from build123d import *

# Parameters (mm, degrees)
SKETCH1_R           = 125
SKETCH1_R_2         = 110
BOSS_EXTRUDE1_DEPTH = 18
SKETCH2_R           = 175
SKETCH2_R_2         = 9
BOSS_EXTRUDE2_DEPTH = 15
CHAMFER1_SIZE       = 2
SKETCH3_R           = 67.5
CUT_EXTRUDE1_DEPTH  = 250.677792364


with BuildPart() as part:
    # Sketch1 → Boss-Extrude1 (new body)
    with BuildSketch(Plane.XY):
        with Locations(Location((0, 0, 0), (0, 0, 180))):
            Circle(SKETCH1_R)
        with Locations(Location((0, 0, 0), (0, 0, 180))):
            Circle(SKETCH1_R_2, mode=Mode.SUBTRACT)
    extrude(amount=BOSS_EXTRUDE1_DEPTH)

    # Sketch2 → Boss-Extrude2 (add)
    with BuildSketch(Plane.XY.offset(18)):
        Circle(SKETCH2_R)
        with Locations((0, 150)):
            Circle(SKETCH2_R_2, mode=Mode.SUBTRACT)
        with Locations((-129.903810568, 75)):
            Circle(SKETCH2_R_2, mode=Mode.SUBTRACT)
        with Locations((-129.903810568, -75)):
            Circle(SKETCH2_R_2, mode=Mode.SUBTRACT)
        with Locations((0, -150)):
            Circle(SKETCH2_R_2, mode=Mode.SUBTRACT)
        with Locations((129.903810568, -75)):
            Circle(SKETCH2_R_2, mode=Mode.SUBTRACT)
        with Locations((129.903810568, 75)):
            Circle(SKETCH2_R_2, mode=Mode.SUBTRACT)
    extrude(amount=BOSS_EXTRUDE2_DEPTH)

    # Chamfer1
    chamfer1_edges = [part.edges().sort_by_distance(p)[0] for p in [
        (-175, 0, 33),
    ]]
    chamfer(chamfer1_edges, length=CHAMFER1_SIZE)

    # Sketch3 → Cut-Extrude1 (cut, through all)
    with BuildSketch(Plane.XY.offset(33)):
        Circle(SKETCH3_R)
    extrude(amount=-CUT_EXTRUDE1_DEPTH, mode=Mode.SUBTRACT)


solid = part.part
Design review of the part built by this model. Coordinates are the model's own, in mm. A direction names the side the tool comes from. Coordinates: 2 decimals unless noted, no trailing zeros. Loops run counter-clockwise (first coordinate to the right, second up) from the corner with the lowest first, then second, coordinate; pieces in that order, holes last. Notation, with made-up numbers: M -16,81 L 36,81 A23 cw 36,97 Z; hole C 63.5,-6 d1. An arc over 180 degrees is marked long. Answer as CSV lines item,"result".
Item 1: For probe 1 along Y at (x, z) = (0, 24); probe 2 along Y at (x, z) = (-1, 6.5); probe 3 along Z at (x, y) = (-152.5, 8), list the stretches that pass through material, from the lowest coordinate up.
Answer list:
probe 1,"-175 to -159, -141 to -67.5, 67.5 to 141, 159 to 175"
probe 2,"-125 to -110, 110 to 125"
probe 3,"18 to 33"
Item 2: Machinability: for faces 1 (the face through (116, 53, 18)), 2 (the face through (74, 2, 33)), which of the approach directions +Z, -Z, +X, -X, +Y, -Y give a long, thin tool a straight path to every point of the face, cutting with its end or side? Answer none if there is none.
Answer list:
face 1,"-Z"
face 2,"+Z, +X, -X, +Y, -Y"
Item 3: The part is to be moulded in two halves that separate along X. For faces 3 (the face through (-137.046, 69.524, 25.395)), 4 (the face through (124.88, -5.5, 8.87)), 5 (the face through (1, 111, 0)), say which applies: pulls with the +X half, pulls with the -X half, needs draft (parallel to the pull), parting line crosses it, or undercut.
Answer list:
face 3,"undercut"
face 4,"parting line crosses it"
face 5,"needs draft"
Item 4: For P1, Ø5, axis at x = 57, z = 14, coming from the -Y side; P2, Ø8, axis at x = 24, z = 3.5, coming from the +Y side; P3, Ø8, axis at x = -95, z = 8, coming from the -Y side, all flat-tipped, find the tip position at first contact; note any pin that passes through.
Answer list:
P1,"y = -112.49"
P2,"y = 123.39"
P3,"y = -85.7"
Item 5: Add section D-D on y = -75. Count the separate pieces of the cut face and the enclosed holes in it, plus the area to 3 significant figures.
Answer list:
separate pieces,"3"
enclosed holes,"0"
area,"4,900 mm²"
Item 6: Add section C-C on x = 0. State the section outline as (y, z) points, plus the area to 3 significant figures.
Answer list:
outline,"M -175,18 L -159,18 L -159,33 L -173,33 L -175,31 Z; M -141,18 L -125,18 L -125,0 L -110,0 L -110,18 L -67.5,18 L -67.5,33 L -141,33 Z; M 67.5,18 L 110,18 L 110,0 L 125,0 L 125,18 L 141,18 L 141,33 L 67.5,33 Z; M 159,18 L 175,18 L 175,31 L 173,33 L 159,33 Z"
area,"3,220 mm²"
Item 7: Add section A-A on z = 26. State the section outline as (x, y) points, plus the area to 3 significant figures.
Answer list:
outline,"C 0,0 d350; hole C -129.9,-75 d18; hole C -129.9,75 d18; hole C 0,0 d135; hole C 0,-150 d18; hole C 0,150 d18; hole C 129.9,-75 d18; hole C 129.9,75 d18"
area,"80,400 mm²"
Item 8: Add section B-B on y = 0. State the section outline as (x, z) points, plus the area to 3 significant figures.
Answer list:
outline,"M -175,18 L -125,18 L -125,0 L -110,0 L -110,18 L -67.5,18 L -67.5,33 L -173,33 L -175,31 Z; M 67.5,18 L 110,18 L 110,0 L 125,0 L 125,18 L 175,18 L 175,31 L 173,33 L 67.5,33 Z"
area,"3,760 mm²"
